```python
from build123d import *

# Parameters (mm, degrees)
BASE_BLOCK_SKETCH_W        = 30
BASE_BLOCK_SKETCH_H        = 50
BASE_BLOCK_DEPTH           = 30
THROUGH_SLOT_SKETCH_W      = 10
THROUGH_SLOT_SKETCH_H      = 35
THROUGH_SLOT_DEPTH         = 60
STEP_NOTCH_SKETCH_W        = 25
STEP_NOTCH_SKETCH_H        = 10
STEP_NOTCH_DEPTH           = 60
NOSE_BOSS_SKETCH_W         = 40
NOSE_BOSS_SKETCH_H         = 30
NOSE_BOSS_DEPTH            = 90
CORNER_CUT_SKETCH_R        = 6
CORNER_CUT_DEPTH           = 60
NOSE_TAPER_30DEG_CUT_DEPTH = 60
SIDE_POCKET_SKETCH_W       = 22.012832553
SIDE_POCKET_SKETCH_H       = 24.1626403
SIDE_POCKET_10MM_DEPTH     = 10
NOSE_PROFILE_CUT_DEPTH     = 30


with BuildPart() as part:
    # Base Block Sketch → Base Block (new, symmetric)
    with BuildSketch(Plane.XY):
        with Locations((15, 25)):
            Rectangle(BASE_BLOCK_SKETCH_W, BASE_BLOCK_SKETCH_H)
    extrude(amount=BASE_BLOCK_DEPTH, both=True)

    # Through Slot Sketch → Through Slot (cut)
    with BuildSketch(Plane(origin=(0, 50, 0), x_dir=(1, 0, 0), z_dir=(0, 1, 0))):
        with Locations((5, 0)):
            Rectangle(THROUGH_SLOT_SKETCH_W, THROUGH_SLOT_SKETCH_H)
    extrude(amount=-THROUGH_SLOT_DEPTH, mode=Mode.SUBTRACT)

    # Step Notch Sketch → Step Notch (cut)
    with BuildSketch(Plane(origin=(30, 0, 0), x_dir=(0, 0, -1), z_dir=(1, 0, 0))):
        with Locations((0, 45)):
            Rectangle(STEP_NOTCH_SKETCH_W, STEP_NOTCH_SKETCH_H)
    extrude(amount=-STEP_NOTCH_DEPTH, mode=Mode.SUBTRACT)

    # Nose Boss Sketch → Nose Boss (add)
    with BuildSketch(Plane(origin=(30, 0, 0), x_dir=(0, 0, -1), z_dir=(1, 0, 0))):
        with Locations((0, 15)):
            Rectangle(NOSE_BOSS_SKETCH_W, NOSE_BOSS_SKETCH_H)
    extrude(amount=NOSE_BOSS_DEPTH)

    # Corner Cut Sketch → Corner Cut (cut)
    with BuildSketch(Plane.XY.offset(20)):
        with Locations((65, 15)):
            Circle(CORNER_CUT_SKETCH_R)
    extrude(amount=-CORNER_CUT_DEPTH, mode=Mode.SUBTRACT)

    # Nose Taper 30deg Sketch → Nose Taper 30deg Cut (cut)
    with BuildSketch(Plane(origin=(0, 30, 0), x_dir=(1, 0, 0), z_dir=(0, 1, 0))):
        Polygon((99.074539678, -20), (120, -20), (120, 0), (99.074539678, -12.08132015), align=None)
        Polygon((99.074539678, 12.08132015), (120, 0), (120, 20), (99.074539678, 20), align=None)
    extrude(amount=-NOSE_TAPER_30DEG_CUT_DEPTH, mode=Mode.SUBTRACT)

    # Side Pocket Sketch → Side Pocket 10mm (cut)
    with BuildSketch(Plane(origin=(0, 30, 0), x_dir=(1, 0, 0), z_dir=(0, 1, 0))):
        with Locations((110.080955955, 0)):
            Rectangle(SIDE_POCKET_SKETCH_W, SIDE_POCKET_SKETCH_H)
    extrude(amount=-SIDE_POCKET_10MM_DEPTH, mode=Mode.SUBTRACT)

    # Nose Profile Sketch → Nose Profile Cut (cut)
    with BuildSketch(Plane(origin=(0, 30, 0), x_dir=(1, 0, 0), z_dir=(0, 1, 0))):
        Polygon((85.358983849, 20), (99.074539678, 12.08132015), (99.074539678, 20), align=None)
        Polygon((99.074539678, -20), (99.074539678, -12.08132015), (85.358983849, -20), align=None)
    extrude(amount=-NOSE_PROFILE_CUT_DEPTH, mode=Mode.SUBTRACT)


solid = part.part
```
Source: CAD feature listing. Evaluate the final solid. Frame: model axes, mm. A direction names the side the tool comes from. Round coordinates to 2 decimals unless told otherwise and drop trailing zeros. Loops run counter-clockwise (first coordinate to the right, second up) from the corner with the lowest first, then second, coordinate; pieces in that order, holes last. Notation, with made-up numbers: M -39,85.25 L -27,85.25 A14 cw -27,93.25 Z; hole C 47,34 d11. An arc over 180 degrees is marked long. Use a Markdown table: item, result. Add a question column.
1. Line query: line 1 (Y direction, x = 65, z = -1); line 2 (Y direction, x = 34, z = -13.5). Output: solid intervals per line, ascending.
2. Section query C-C on z = 8. Return the cut outline in (x, y), then the cut area to 3 significant figures.
3. Reachability of faces 4 (the flat face through (57, 15, 20)), 5 (the flat face through (5, 25, -17.5)), 6 (the flat face through (107, 20, 0)) from +Z, -Z, +X, -X, +Y, -Y: full face, straight path, thin tool, end or side. Return the list, or none.
4. Contact query for flat-ended pins moving along their axis: P1, Ø10.5, axis at y = 17.5, z = 5.5, coming from the -X side; P2, Ø12, axis at x = 50.5, z = -0.5, coming from the +Y side; P3, Ø8, axis at x = 66.5, y = 7.5, coming from the +Z side; P4, Ø3, axis at x = 38, y = 33, coming from the -Z side (3 decimals). Output: stop coordinate, or through.
5. Section query D-D on y = 15. Return the cut outline in (x, z).
6. Section query B-B on x = 65. Return the cut outline in (y, z).
7. Mould query, pull axis Z, two halves, no side actions, for faces 1 (the flat face through (20, 40, 0)), 2 (the flat face through (15, 50, 21)), 3 (the flat face through (15, 25, -30)). Classes: pulls with the +Z half, pulls with the -Z half, needs draft (parallel to the pull), parting line crosses it, or undercut.
8. Section query A-A on y = 42.5. Return the cut outline in (x, z), then the cut area to 3 significant figures.
Reported:
| question | item | result |
|---|---|---|
| 1 | line 1 | y = 0 to 9, 21 to 30 |
| 1 | line 2 | y = 0 to 30 |
| 2 | outline | M 10,0 L 106.14,0 L 106.14,20 L 99.07,20 L 99.07,30 L 30,30 L 30,40 L 10,40 Z; hole C 65,15 d12 |
| 2 | area | 2,900 mm² |
| 3 | face 4 | +Z, +X, +Y, -Y |
| 3 | face 5 | -X, +Y, -Y |
| 3 | face 6 | +Z, -Z, +X, +Y |
| 4 | P1 | stops at x = 10 |
| 4 | P2 | stops at y = 30 |
| 4 | P3 | stops at z = 20 |
| 4 | P4 | passes through |
| 5 | outline | M 0,-30 L 30,-30 L 30,-20 L 59,-20 L 59,20 L 30,20 L 30,30 L 0,30 L 0,17.5 L 10,17.5 L 10,-17.5 L 0,-17.5 Z; M 71,-20 L 85.36,-20 L 120,0 L 85.36,20 L 71,20 Z |
| 6 | outline | M 0,-20 L 9,-20 L 9,20 L 0,20 Z; M 21,-20 L 30,-20 L 30,20 L 21,20 Z |
| 7 | face 1 | undercut |
| 7 | face 2 | needs draft |
| 7 | face 3 | pulls with the -Z half |
| 8 | outline | M 0,-30 L 30,-30 L 30,-12.5 L 10,-12.5 L 10,-17.5 L 0,-17.5 Z; M 0,17.5 L 10,17.5 L 10,12.5 L 30,12.5 L 30,30 L 0,30 Z |
| 8 | area | 950 mm² |
